```python
from build123d import *

# Parameters (mm, degrees)
SKETCH1_W           = 60
SKETCH1_H           = 80
SKETCH1_R           = 3
BOSS_EXTRUDE1_DEPTH = 3
SKETCH2_R           = 5
CUT_EXTRUDE1_DEPTH  = 3


with BuildPart() as part:
    # Sketch1 → Boss-Extrude1 (new body)
    with BuildSketch(Plane(origin=(0, 0, 0), x_dir=(0, 0, -1), z_dir=(1, 0, 0))):
        Rectangle(SKETCH1_W, SKETCH1_H)
        with Locations((-25, 20)):
            Circle(SKETCH1_R, mode=Mode.SUBTRACT)
        with Locations((0, -10)):
            Circle(SKETCH1_R, mode=Mode.SUBTRACT)
    extrude(amount=BOSS_EXTRUDE1_DEPTH)

    # Sketch2 → Cut-Extrude1 (cut)
    with BuildSketch(Plane(origin=(3, 0, 0), x_dir=(0, 0, -1), z_dir=(1, 0, 0))):
        with Locations((0, -10)):
            Circle(SKETCH2_R)
    extrude(amount=-CUT_EXTRUDE1_DEPTH, mode=Mode.SUBTRACT)


solid = part.part
```
Geometry: final body of the model. Coordinates: model frame, mm. Coordinates: 2 decimals unless noted, no trailing zeros. Loops run counter-clockwise (first coordinate to the right, second up) from the corner with the lowest first, then second, coordinate; pieces in that order, holes last. Notation, with made-up numbers: M 66.5,75.5 L 112.5,75.5 A14 ccw 112.5,100.5 Z; hole C 67.5,24.5 d4. An arc over 180 degrees is marked long. Put each result on its own line as item: value.
(1) Cut plane C-C on x = 2.35. Return the cut outline in (y, z).
Answer sheet:
outline: M -40,-30 L 40,-30 L 40,30 L -40,30 Z; hole C -10,0 d10; hole C 20,25 d6
(2) Draft query along Z for faces 1 (the face through (1, -40, 0)), 2 (the face through (1.5, 18.2, 27.4)), 3 (the face through (1, -1, -30)), 4 (the face through (1, -1, 30)). Return one class per face: pulls with the +Z half, pulls with the -Z half, needs draft (parallel to the pull), parting line crosses it, or undercut.
Answer sheet:
face 1: needs draft
face 2: undercut
face 3: pulls with the -Z half
face 4: pulls with the +Z half
(3) Cut plane B-B on y = 20. Return the cut outline in (x, z), then the cut area to 3 significant figures.
Answer sheet:
outline: M 0,-30 L 3,-30 L 3,22 L 0,22 Z; M 0,28 L 3,28 L 3,30 L 0,30 Z
area: 162 mm^2
(4) Material intervals for probe 1 along Y at (x, z) = (2.05, 25); probe 2 along Y at (x, z) = (1.8, 0), sorted ascending.
Answer sheet:
probe 1: y = -40 to 17, 23 to 40
probe 2: y = -40 to -15, -5 to 40
(5) Cut plane A-A on z = 25. Return the cut outline in (x, y).
Answer sheet:
outline: M 0,-40 L 3,-40 L 3,17 L 0,17 Z; M 0,23 L 3,23 L 3,40 L 0,40 Z
(6) First-contact query: pin 1 (1 mm diameter, centred on y = 15.5, z = 18, fed in from -X). Flat tip, straight axial feed; report the tip coordinate or a pass-through.
Answer sheet:
pin 1: stops at x = 0
